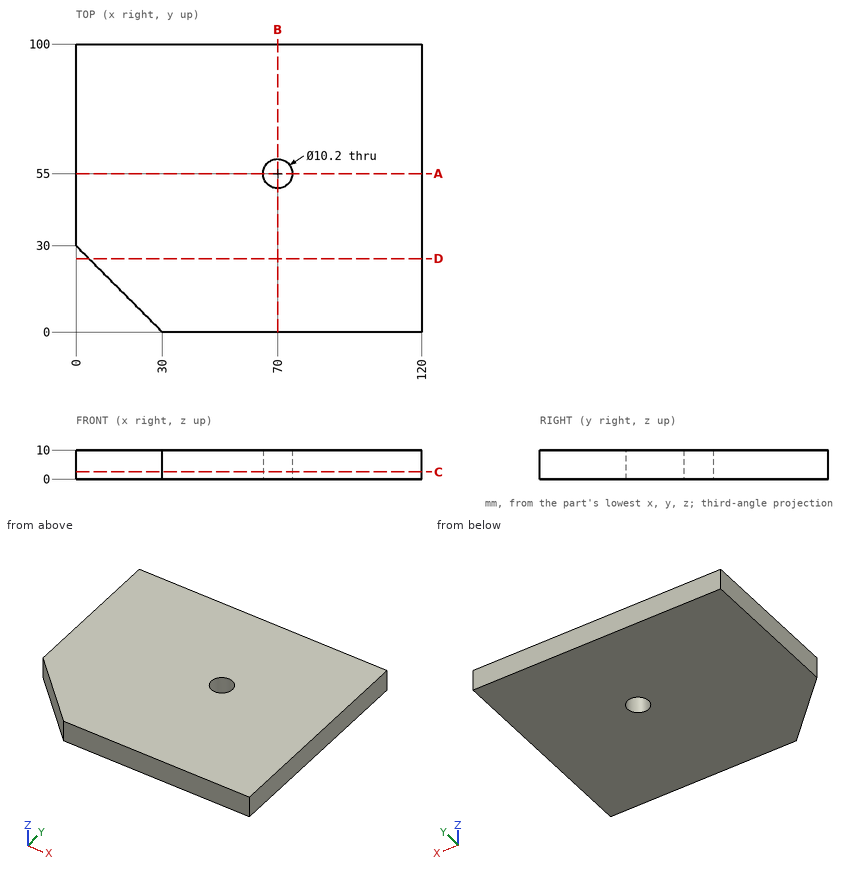
Here's the drawing with two shaded views (mm, measured from the low corner). I have some questions. Round coordinates to 2 decimals unless told otherwise and drop trailing zeros. Loops run counter-clockwise (first coordinate to the right, second up) from the corner with the lowest first, then second, coordinate; pieces in that order, holes last.
1. Suppose I cut it at D-D, the plane y = 25.5. Please give me the cut outline in (x, z).
Answers:
outline: (4.5, 0) - (120, 0) - (120, 10) - (4.5, 10) - close
2. If I drill on probe 1 along Y at (x, z) = (70, 7.75); probe 2 along X at (y, z) = (57, 3.25); probe 3 along Y at (x, z) = (15, 9.25), over which ranges is the centre line in solid material (lowest first)?
Answers:
probe 1: y = 0 to 49.9, 60.1 to 100
probe 2: x = 0 to 65.31, 74.69 to 120
probe 3: y = 15 to 100
3. Suppose I cut it at A-A, the plane y = 55. Please give me the cut outline in (x, z).
Answers:
outline: (0, 0) - (64.9, 0) - (64.9, 10) - (0, 10) - close; (75.1, 0) - (120, 0) - (120, 10) - (75.1, 10) - close
4. Suppose I cut it at B-B, the plane x = 70. Please give me the cut outline in (y, z).
Answers:
outline: (0, 0) - (49.9, 0) - (49.9, 10) - (0, 10) - close; (60.1, 0) - (100, 0) - (100, 10) - (60.1, 10) - close
5. Suppose I cut it at C-C, the plane z = 2.5. Please give me the cut outline in (x, y).
Answers:
outline: (0, 30) - (30, 0) - (120, 0) - (120, 100) - (0, 100) - close; hole circle Ø10.2 at (70, 55)
